from build123d import *

# Parameters (mm, degrees)
SKETCH_1_R               = 8
EXTRUDE_1_DEPTH          = 13
CUT_EXTRUDE_2_DEPTH      = 23.472205054
PATTERN_CIRCULAR_1_COUNT = 3
SKETCH_2_R               = 9.3675
SKETCH_2_R_2             = 8
EXTRUDE_2_DEPTH          = 1.8
SKETCH_4_OUTSIDE_W       = 208.978
SKETCH_4_OUTSIDE_H       = 212.69
SKETCH_4_OUTSIDE_R       = 12
CUT_EXTRUDE_3_DEPTH      = 23.472205054
CUT_EXTRUDE_3_DRAFT      = -75
SKETCH_5_R               = 9.565
CUT_EXTRUDE_4_DEPTH      = 0.2


with BuildPart() as part:
    # 草图1 → 拉伸1 (new body)
    with BuildSketch(Plane.XY):
        Polygon((0, 13.856406461), (-12, 6.92820323), (-12, -6.92820323), (0, -13.856406461), (12, -6.92820323), (12, 6.92820323), align=None)
        with Locations(Location((0, 0, 0), (0, 0, 180))):
            Circle(SKETCH_1_R, mode=Mode.SUBTRACT)
    extrude(amount=EXTRUDE_1_DEPTH)

    # 草图3 → 切除-拉伸2 (cut, symmetric)
    with BuildSketch(Plane(origin=(0, 0, 0), x_dir=(0, 0, -1), z_dir=(1, 0, 0))):
        Polygon((-12.2, 12.133037667), (-11.2, 11.666730008), (-11.2, 0), (-13, 0), (-13, 13.856406461), (-12.2, 13.856406461), align=None)
    cut_extrude_2 = extrude(amount=CUT_EXTRUDE_2_DEPTH, both=True, mode=Mode.SUBTRACT)

    # 阵列(圆周)1: 切除-拉伸2 ×3 about axis
    pattern_circular_1_axis = Axis((0, 0, 0), (0, 0, 1))
    for i in range(1, PATTERN_CIRCULAR_1_COUNT):
        add(cut_extrude_2.rotate(pattern_circular_1_axis, i * 360 / PATTERN_CIRCULAR_1_COUNT), mode=Mode.SUBTRACT)

    # 草图2 → 拉伸2 (add)
    with BuildSketch(Plane.XY.offset(11.2)):
        with Locations(Location((0, 0, 0), (0, 0, 180))):
            Circle(SKETCH_2_R)
        with Locations(Location((0, 0, 0), (0, 0, 180))):
            Circle(SKETCH_2_R_2, mode=Mode.SUBTRACT)
    extrude(amount=EXTRUDE_2_DEPTH)


with BuildPart() as cut_extrude_3_tool:
    # 草图4 outside → 切除-拉伸3 (with draft: the straight prism first)
    with BuildSketch(Plane(origin=(0, 0, 0), x_dir=(-1, 0, 0), z_dir=(0, 0, -1))):
        Rectangle(SKETCH_4_OUTSIDE_W, SKETCH_4_OUTSIDE_H)
        Circle(SKETCH_4_OUTSIDE_R, mode=Mode.SUBTRACT)
    extrude(amount=-CUT_EXTRUDE_3_DEPTH)
    # 切除-拉伸3: the draft: its side faces are tilted about the plane it starts from
    cut_extrude_3_sides = [cut_extrude_3_tool.faces().sort_by_distance(p)[0] for p in [
        (0, -106.345, 11.736102527),
        (-104.489, 0, 11.736102527),
        (0, 106.345, 11.736102527),
        (104.489, 0, 11.736102527),
        (12, 0, 11.736102527),
    ]]
    draft(cut_extrude_3_sides, Plane(origin=(0, 0, 0), x_dir=(-1, 0, 0), z_dir=(0, 0, -1)), CUT_EXTRUDE_3_DRAFT)


with BuildPart() as part_1:
    add(part.part)

    # 切除-拉伸3: cut by cut_extrude_3_tool
    add(cut_extrude_3_tool.part, mode=Mode.SUBTRACT)

    # 草图5 → 切除-拉伸4 (cut)
    with BuildSketch(Plane(origin=(0, 0, 0), x_dir=(-1, 0, 0), z_dir=(0, 0, -1))):
        Circle(SKETCH_5_R)
    extrude(amount=-CUT_EXTRUDE_4_DEPTH, mode=Mode.SUBTRACT)


solid = part_1.part
CAD build for the part. Positions are in the model's coordinates, mm. A direction names the side the tool comes from. Round coordinates to 2 decimals unless told otherwise and drop trailing zeros. Write each loop counter-clockwise with the first axis right and the second up, starting at its lowest first coordinate (ties: lowest second). Pieces come first, ordered by that corner, then holes.
(1) Probe line 1 along X through (y, z) = (0.25, 3.5); line 2 along X through (y, z) = (5.25, 7.25); line 3 along Y through (x, z) = (4.75, 8.75). List the from-to ranges inside material, lowest first.
(2) Slice it at A-A, the plane z = 5.25. Write the cut outline in (x, y), and give its area (3 significant figures).
(3) 3-axis set-ups, long thin cutter, end or side, ignore diameter. For faces 1 (the face through (-8, -3, 13)), 2 (the face through (0, 13, 12.2)), 3 (the face through (10.28, -6, 11.71)), 4 (the face through (2, -8, 0.2)): which of +Z, -Z, +X, -X, +Y, -Y reach the whole face in a straight line?
(4) Mould opens along Y. For faces 5 (the face through (0.1, 11.9, 11.7)), 6 (the face through (-10.791, 6.195, 0.119)), 7 (the face through (0.03, -12.443, 0.119)) say: pulls with the +Y half, pulls with the -Y half, needs draft (parallel to the pull), parting line crosses it, or undercut.
(5) Drop flat-ended pins along their axis: P1, Ø1.5, axis at x = -1, y = -9.5, coming from the +Z side; P2, Ø1.4, axis at x = 1, y = 13.5, coming from the +Z side; P3, Ø4, axis at x = -7, z = 3.5, coming from the -Y side; P4, Ø3, axis at x = -3, z = 9, coming from the -Y side. Give the stop position or say it passes through.
From the geometry:
1. line 1: x = -12 to -8, 8 to 12
1. line 2: x = -12 to -6.04, 6.04 to 12
1. line 3: y = -11.11 to -6.44, 6.44 to 11.11
2. outline: (-12, -6.93) - (0, -13.86) - (12, -6.93) - (12, 6.93) - (0, 13.86) - (-12, 6.93) - close; hole circle Ø16 at (0, 0)
2. area: 298 mm2
3. face 1: +Z, +X, -X, +Y, -Y
3. face 2: +Z, +X, -X, +Y
3. face 3: +Z
3. face 4: -Z
4. face 5: undercut
4. face 6: pulls with the +Y half
4. face 7: pulls with the -Y half
5. P1: stops at z = 13
5. P2: stops at z = 12.2
5. P3: stops at y = -10.97
5. P4: stops at y = -12.99
